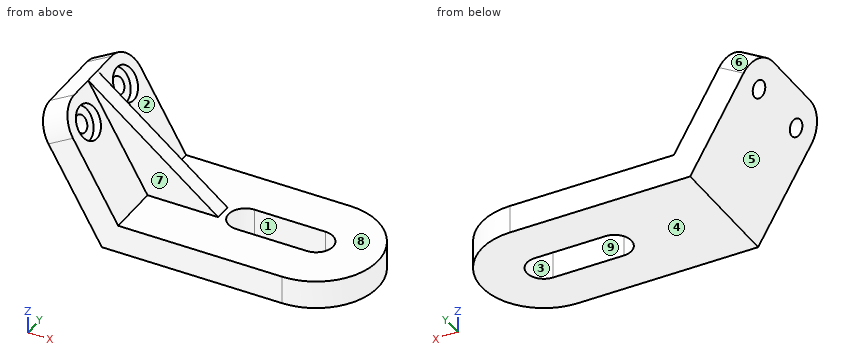
from build123d import *

# Parameters (mm, degrees)
BASE_PLATE_SKETCH_W        = 58
BASE_PLATE_SKETCH_H        = 44
BASE_PLATE_58X44X10_DEPTH  = 10
BASE_ROUNDED_END_SKETCH_R  = 22
BASE_ROUNDED_END_R22_DEPTH = 10
BASE_SLOT_DEPTH            = 10
ANGLED_ARM_120DEG_DEPTH    = 44
ARM_END_TRIM_DEPTH         = 10
COUNTERBORE_SKETCH_R       = 6
COUNTERBORES_2X_12X3_DEPTH = 3
ARM_HOLE_SKETCH_R          = 3
ARM_HOLES_2X_6_DEPTH       = 10
GUSSET_BLANK_DEPTH         = 44
GUSSET_SIDE_TRIM_1_DEPTH   = 19
GUSSET_SIDE_TRIM_2_DEPTH   = 19


with BuildPart() as part:
    # Base Plate Sketch → Base Plate 58x44x10 (new body)
    with BuildSketch(Plane.XY):
        with Locations((29, 22)):
            Rectangle(BASE_PLATE_SKETCH_W, BASE_PLATE_SKETCH_H)
    extrude(amount=BASE_PLATE_58X44X10_DEPTH)

    # Base Rounded End Sketch → Base Rounded End R22 (add)
    with BuildSketch(Plane.XY.offset(10)):
        with Locations((58, 22)):
            Circle(BASE_ROUNDED_END_SKETCH_R)
    extrude(amount=-BASE_ROUNDED_END_R22_DEPTH)

    # Base Slot Sketch → Base Slot (cut)
    with BuildSketch(Plane.XY.offset(10)):
        with BuildLine():
            Line((33, 28), (58, 28))
            ThreePointArc((58, 28), (64, 22), (58, 16))
            Line((58, 16), (33, 16))
            ThreePointArc((33, 16), (27, 22), (33, 28))
        make_face()
    extrude(amount=-BASE_SLOT_DEPTH, mode=Mode.SUBTRACT)

    # Angled Arm Sketch → Angled Arm 120deg (add)
    with BuildSketch(Plane.XZ):
        Polygon((-29.660254038, 41.373066959), (-5.773502692, 0), (0, 0), (0, 10), (-21, 46.373066959), align=None)
    extrude(amount=-ANGLED_ARM_120DEG_DEPTH)

    # Arm End Trim Sketch → Arm End Trim (cut)
    with BuildSketch(Plane(origin=(4.330127019, 0, 2.5), x_dir=(0.5000000000000042, 0, -0.8660254037844363), z_dir=(0.8660254037844363, 0, 0.5000000000000042))):
        with BuildLine():
            Line((-50.660254038, 0), (-40.660254038, 0))
            ThreePointArc((-40.660254038, 0), (-47.73132185, 2.928932188), (-50.660254038, 10))
            Line((-50.660254038, 10), (-50.660254038, 0))
        make_face()
        with BuildLine():
            Line((-50.660254038, 44), (-40.660254038, 44))
            ThreePointArc((-40.660254038, 44), (-47.73132185, 41.071067812), (-50.660254038, 34))
            Line((-50.660254038, 34), (-50.660254038, 44))
        make_face()
    extrude(amount=-ARM_END_TRIM_DEPTH, mode=Mode.SUBTRACT)

    # Counterbore Sketch → Counterbores 2xØ12x3 (cut)
    with BuildSketch(Plane(origin=(4.330127019, 0, 2.5), x_dir=(0.5000000000000042, 0, -0.8660254037844363), z_dir=(0.8660254037844363, 0, 0.5000000000000042))):
        with Locations((-40.660254038, 34)):
            Circle(COUNTERBORE_SKETCH_R)
        with Locations((-40.660254038, 10)):
            Circle(COUNTERBORE_SKETCH_R)
    extrude(amount=-COUNTERBORES_2X_12X3_DEPTH, mode=Mode.SUBTRACT)

    # Arm Hole Sketch → Arm Holes 2xØ6 (cut)
    with BuildSketch(Plane(origin=(1.732050808, 0, 1), x_dir=(0.5000000000000042, 0, -0.8660254037844363), z_dir=(0.8660254037844363, 0, 0.5000000000000042))):
        with Locations((-40.660254038, 34)):
            Circle(ARM_HOLE_SKETCH_R)
        with Locations((-40.660254038, 10)):
            Circle(ARM_HOLE_SKETCH_R)
    extrude(amount=-ARM_HOLES_2X_6_DEPTH, mode=Mode.SUBTRACT)

    # Gusset Profile Sketch → Gusset Blank (add)
    with BuildSketch(Plane.XZ):
        Polygon((0, 10), (25, 10), (-21, 46.373066959), align=None)
    extrude(amount=-GUSSET_BLANK_DEPTH)

    # Gusset Side Trim 1 Sketch → Gusset Side Trim 1 (cut)
    with BuildSketch(Plane.XZ):
        Polygon((4.891585761, 10), (25, 10), (-21, 46.373066959), (0, 10), align=None)
    extrude(amount=-GUSSET_SIDE_TRIM_1_DEPTH, mode=Mode.SUBTRACT)

    # Gusset Side Trim 2 Sketch → Gusset Side Trim 2 (cut)
    with BuildSketch(Plane(origin=(0, 44, 0), x_dir=(1, 0, 0), z_dir=(0, 1, 0))):
        Polygon((25, -10), (0, -10), (-21, -46.373066959), align=None)
    extrude(amount=-GUSSET_SIDE_TRIM_2_DEPTH, mode=Mode.SUBTRACT)


solid = part.part
Source: CAD feature listing. Evaluate the final solid. Frame: model axes, mm. Face numbers are marked on the shaded views. A direction names the side the tool comes from. Give positions to 0.01 mm unless a question says otherwise; leave off trailing zeros. Write each loop counter-clockwise with the first axis right and the second up, starting at its lowest first coordinate (ties: lowest second). Pieces come first, ordered by that corner, then holes. Notation, with made-up numbers: M 50.25,71 L 101.25,71 A13 cw 101.25,93 Z; hole C 44,23 d9. An arc over 180 degrees is marked long. Return JSON: item names as keys, results as strings. Group by question number.
1) Cut plane D-D, the plane z = 14.5. Output: boundary loops of the cut face in (x, y), then the cut area to 3 significant figures.
2) First-contact query: pin 1 Ø12 at (y, z) = (5.5, 17) entering from -X; pin 2 Ø2 at (x, z) = (5, 16) entering from +Y; pin 3 Ø22 at (x, y) = (29, 11.5) entering from +Z. Flat tips, straight axial feed; report the tip coordinate or a pass-through.
3) Cut plane B-B, the plane x = 39. Output: boundary loops of the cut face in (y, z).
4) Cut plane A-A, the plane y = 22. Output: boundary loops of the cut face in (x, z), then the cut area to 3 significant figures.
5) Set-up query: the marked faces 5, 6, 7, 8 and 9. Return all of +Z, -Z, +X, -X, +Y, -Y with unobstructed straight access to the full face (end or side cutting, diameter ignored); none if empty.
6) Draft query along X for the marked faces 1, 2, 3 and 4. Return one class per face: released by +X, released by -X, zero draft, split by the parting line, or undercut.
7) Ray query, L1, parallel to Y at x = 48.5, z = 5; L2, parallel to Z at x = 38, y = 32; L3, parallel to Y at x = 13.5, z = 15. Return the intervals inside material, ascending.
8) Cut plane C-C, the plane z = 4.5. Output: boundary loops of the cut face in (x, y), then the cut area to 3 significant figures.
Data:
{
 "1": {"outline": "M -14.15,0 L -2.6,0 L -2.6,19 L 19.31,19 L 19.31,25 L -2.6,25 L -2.6,44 L -14.15,44 Z", "area": "640 mm²"},
 "2": {"pin 1": "stops at x = -19.05", "pin 2": "stops at y = 25", "pin 3": "stops at z = 13.2"},
 "3": {"outline": "M 0,0 L 16,0 L 16,10 L 0,10 Z; M 28,0 L 44,0 L 44,10 L 28,10 Z"},
 "4": {"outline": "M -29.66,41.37 L -5.77,0 L 27,0 L 27,10 L 25,10 L -21,46.37 Z; M 64,0 L 80,0 L 80,10 L 64,10 Z", "area": "1,360 mm²"},
 "5": {"face 5": "-Z, -X, +Y, -Y", "face 6": "+Z, -X, +Y", "face 7": "+Z, +X, -Y", "face 8": "+Z, +X", "face 9": "+Z, -Z"},
 "6": {"face 1": "undercut", "face 2": "released by +X", "face 3": "undercut", "face 4": "zero draft"},
 "7": {"L1": "y = 0 to 16, 28 to 44", "L2": "z = 0 to 10", "L3": "y = 19 to 25"},
 "8": {"outline": "M -8.37,0 L 58,0 A22 ccw 58,44 L -8.37,44 Z; hole M 33,16 L 58,16 A6 ccw 58,28 L 33,28 A6 ccw Z", "area": "3,270 mm²"}
}
